```python
from build123d import *


with BuildPart() as part:
    # Sketch1 → Revolve1 (revolve)
    with BuildSketch(Plane.XY, mode=Mode.PRIVATE) as revolve1_sk:
        Polygon((70, 0), (80, 0), (80, -5), (85, -5), (85, -26), (65, -26), (65, -21), (67.5, -21), (67.5, -12.5), (69, -12.5), (69, -7.5), (72, -7.5), (72, -3), (70, -3), align=None)
    revolve(revolve1_sk.sketch.rotate(Axis((0, 0, 0), (0, -1, 0)), 90), axis=Axis((0, 0, 0), (0, -1, 0)))


solid = part.part
```
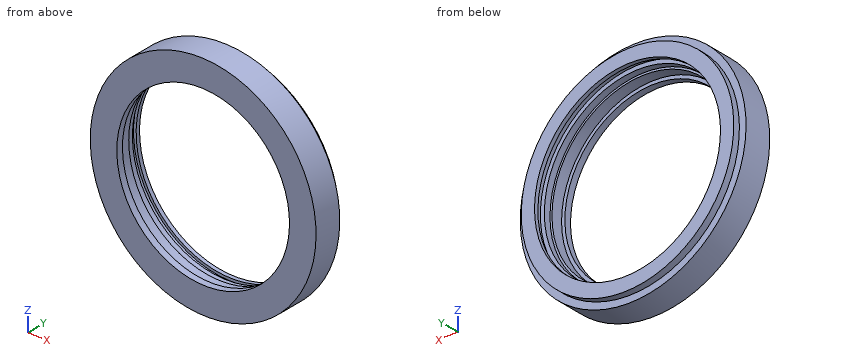
Geometry: final body of the model. Coordinates: model frame, mm. Coordinates: 2 decimals unless noted, no trailing zeros. Order: outer loops, then holes, each group sorted by start corner. A loop starts at its lowest first (then second) coordinate and runs counter-clockwise, first axis right, second up. Notation, with made-up numbers: (86, 74) - (144, 74) arc R26 cw to (144, 110) - close; hole circle Ø11 at (28.25, -11). An arc over 180 degrees is marked (long way). Write each question's results on one line, items separated by ' | '.
(1) Section query D-D, the plane z = -75. Return the cut outline in (x, y), plus the area to 3 significant figures.
Values found:
outline: (-40, -26) - (40, -26) - (40, -5) - (27.84, -5) - (27.84, 0) - (-27.84, 0) - (-27.84, -5) - (-40, -5) - close | area: 1,960 mm²
(2) Section query B-B, the plane z = 0. Return the cut outline in (x, y).
Values found:
outline: (-85, -26) - (-65, -26) - (-65, -21) - (-67.5, -21) - (-67.5, -12.5) - (-69, -12.5) - (-69, -7.5) - (-72, -7.5) - (-72, -3) - (-70, -3) - (-70, 0) - (-80, 0) - (-80, -5) - (-85, -5) - close; (65, -26) - (85, -26) - (85, -5) - (80, -5) - (80, 0) - (70, 0) - (70, -3) - (72, -3) - (72, -7.5) - (69, -7.5) - (69, -12.5) - (67.5, -12.5) - (67.5, -21) - (65, -21) - close
(3) Line query: line 1 (X direction, y = -11.05, z = 0); line 2 (Z direction, x = -1, y = -24); line 3 (X direction, y = -16, z = 0). Output: solid intervals per line, ascending. Write a range as [from, to].
Values found:
line 1: x = [-85, -69], [69, 85] | line 2: z = [-84.99, -64.99], [64.99, 84.99] | line 3: x = [-85, -67.5], [67.5, 85]
(4) Section query C-C, the plane y = -18. Return the cut outline in (x, z), plus the area to 3 significant figures.
Values found:
outline: circle Ø170 at (0, 0); hole circle Ø135 at (0, 0) | area: 8,380 mm²
(5) Section query A-A, the plane x = 0. Return the cut outline in (y, z).
Values found:
outline: (-26, -85) - (-5, -85) - (-5, -80) - (0, -80) - (0, -70) - (-3, -70) - (-3, -72) - (-7.5, -72) - (-7.5, -69) - (-12.5, -69) - (-12.5, -67.5) - (-21, -67.5) - (-21, -65) - (-26, -65) - close; (-26, 65) - (-21, 65) - (-21, 67.5) - (-12.5, 67.5) - (-12.5, 69) - (-7.5, 69) - (-7.5, 72) - (-3, 72) - (-3, 70) - (0, 70) - (0, 80) - (-5, 80) - (-5, 85) - (-26, 85) - close
(6) First-contact query: pin 1 Ø8 at (x, y) = (-29.5, -22) entering from +Z; pin 2 Ø1.5 at (x, y) = (2.5, -20.5) entering from +Z; pin 3 Ø1 at (y, z) = (-17, 10) entering from +X. Flat tips, straight axial feed; report the tip coordinate or a pass-through.
Values found:
pin 1: stops at z = 81.08 | pin 2: stops at z = 84.98 | pin 3: stops at x = 84.47
